from build123d import *

# Parameters (mm, degrees)
EXTRUDE_THIN1_DEPTH = 480


with BuildPart() as part:
    # Sketch1 → Extrude-Thin1 (new body)
    with BuildSketch(Plane.XY):
        with BuildLine():
            Line((0, -115.5), (0, -10))
            ThreePointArc((0, -10), (2.928932188, -2.928932188), (10, 0))
            Line((10, 0), (526, 0))
            ThreePointArc((526, 0), (533.071067812, -2.928932188), (536, -10))
            Line((536, -10), (536, -115.5))
            Line((536, -115.5), (534, -115.5))
            Line((534, -115.5), (534, -10))
            ThreePointArc((534, -10), (531.656854249, -4.343145751), (526, -2))
            Line((526, -2), (10, -2))
            ThreePointArc((10, -2), (4.343145751, -4.343145751), (2, -10))
            Line((2, -10), (2, -115.5))
            Line((2, -115.5), (0, -115.5))
        make_face()
    extrude(amount=EXTRUDE_THIN1_DEPTH)


solid = part.part
Work out the finished part from the listing and answer in its coordinate system (mm). A direction names the side the tool comes from. Coordinates: 2 decimals unless noted, no trailing zeros. Loops run counter-clockwise (first coordinate to the right, second up) from the corner with the lowest first, then second, coordinate; pieces in that order, holes last. Notation, with made-up numbers: M -2.5,-37.75 L 15.5,-37.75 A8 ccw 15.5,-27.75 Z; hole C -35,86.25 d7. An arc over 180 degrees is marked long. Answer in a Markdown table with one row per item. Add a question column.
1. Consider L1, parallel to X at y = -104, z = 240; L2, parallel to Y at x = 320, z = 111. Determine where each line is inside the solid, lowest interval first.
2. A tool of negligible diameter and unlimited length cuts with its end or side. For faces 5 (the flat face through (536, -62, 237)), 6 (the flat face through (534, -63, 237)), from which of +Z, -Z, +X, -X, +Y, -Y can it reach the whole face along a straight path? Write none if from no direction.
3. The mould has two halves that part along X. Classify faces 1 (the flat face through (0, -63, 237)), 2 (the flat face through (272, -2, 237)), 3 (the flat face through (2, -62, 237)), 4 (the flat face through (264, 0, 237)): pulls with the +X half, pulls with the -X half, needs draft (parallel to the pull), parting line crosses it, or undercut.
4. Find section A-A, the plane y = -55.5. Write down the section's boundary in (x, z), then the cut area to 3 significant figures.
5. Find section C-C, the plane x = 243. Write down the section's boundary in (y, z), then the cut area to 3 significant figures.
6. A flat-ended cylindrical pin translates along its axis: P1, Ø5, axis at x = 120.5, z = 57, coming from the -Y side. Find the tip coordinate at first contact, or state that the pin passes through.
7. Find section B-B, the plane z = 240.5. Write down the section's boundary in (x, y).
Reported:
| question | item | result |
|---|---|---|
| 1 | L1 | x = 0 to 2, 534 to 536 |
| 1 | L2 | y = -2 to 0 |
| 2 | face 5 | +Z, -Z, +X, +Y, -Y |
| 2 | face 6 | +Z, -Z, -Y |
| 3 | face 1 | pulls with the -X half |
| 3 | face 2 | undercut |
| 3 | face 3 | undercut |
| 3 | face 4 | needs draft |
| 4 | outline | M 0,0 L 2,0 L 2,480 L 0,480 Z; M 534,0 L 536,0 L 536,480 L 534,480 Z |
| 4 | area | 1,920 mm^2 |
| 5 | outline | M -2,0 L 0,0 L 0,480 L -2,480 Z |
| 5 | area | 960 mm^2 |
| 6 | P1 | stops at y = -2 |
| 7 | outline | M 0,-115.5 L 2,-115.5 L 2,-10 A8 cw 10,-2 L 526,-2 A8 cw 534,-10 L 534,-115.5 L 536,-115.5 L 536,-10 A10 ccw 526,0 L 10,0 A10 ccw 0,-10 Z |
